The model under review builds one solid part; all positions refer to its coordinate system, in mm. Face numbers are marked on the shaded views. A direction names the side the tool comes from. Round coordinates to 2 decimals unless told otherwise and drop trailing zeros. Order: outer loops, then holes, each group sorted by start corner. A loop starts at its lowest first (then second) coordinate and runs counter-clockwise, first axis right, second up. Notation, with made-up numbers: M 42,29.5 L 57,29.5 A19 cw 57,56.5 Z; hole C -27,43 d8. An arc over 180 degrees is marked long. Answer as a JSON object with one key per item and string values. Group by question number.
1) For the marked faces 1, 2, 3 and 4, list the 3-axis set-ups (+Z, -Z, +X, -X, +Y, -Y) from which the entire face can be reached by the end or side of a thin tool; tool diameter is ignored.
2) The part is to be moulded in two halves that separate along X. For the marked faces 5, 6, 7 and 8, say which applies: +X half, -X half, draft (parallel to the pull), parting line (faces both ways), or undercut.
3) Insertion check: pin 1 Ø10 at (y, z) = (51, 35) entering from +X; pin 2 Ø1.5 at (y, z) = (25.5, 29) entering from +X; pin 3 Ø12 at (x, y) = (45, 34) entering from +Z; pin 4 Ø16 at (y, z) = (40.5, 29.5) entering from -X. Each pin has a flat end and moves straight along its axis. Give the tip position at first contact, or say it passes through.
4) To check wall thickness, follow line 1 (X direction, y = 36.5, z = 26); line 2 (Y direction, x = 50, z = 16.25); line 3 (Z direction, x = 95.5, y = 27). State the ranges of each line that lie inside material, in increasing order.
5) Consider section C-C, the plane z = 32. Write out the cut boundary in (x, y), then the cut area to 3 significant figures.
6) Consider section D-D, the plane y = 45. Write out the cut boundary in (x, z).
7) Consider section B-B, the plane y = 30. Write out the cut boundary in (x, z), then the cut area to 3 significant figures.
8) Consider section A-A, the plane x = 50. Write out the cut boundary in (y, z), then the cut area to 3 significant figures.
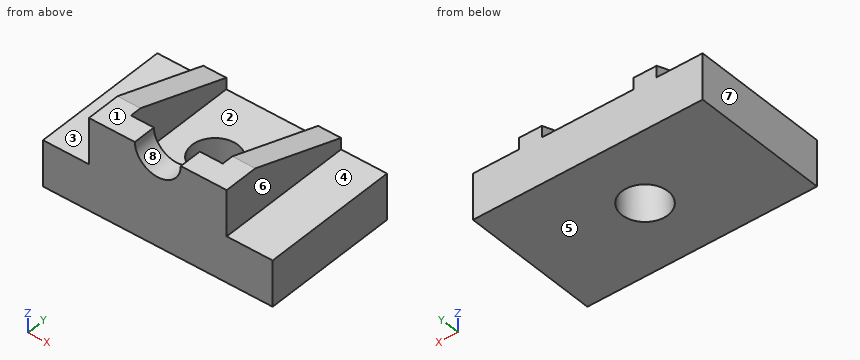
```python
from build123d import *

# Parameters (mm, degrees)
BACK_PLATE_SKETCH_W       = 100
BACK_PLATE_SKETCH_H       = 60
BACK_PLATE_DEPTH          = 20
BORE_20_SKETCH_R          = 10
BORE_20_DEPTH             = 20
NOTCHED_BASE_FLANGE_DEPTH = 10
LEFT_GUSSET_DEPTH         = 10
RIGHT_GUSSET_DEPTH        = 10


with BuildPart() as part:
    # Back Plate Sketch → Back Plate (new body)
    with BuildSketch(Plane.XY):
        with Locations((50, 30)):
            Rectangle(BACK_PLATE_SKETCH_W, BACK_PLATE_SKETCH_H)
    extrude(amount=BACK_PLATE_DEPTH)

    # Bore Ø20 Sketch → Bore Ø20 (cut)
    with BuildSketch(Plane.XY.offset(20)):
        with Locations((50, 30)):
            Circle(BORE_20_SKETCH_R)
    extrude(amount=-BORE_20_DEPTH, mode=Mode.SUBTRACT)

    # Base Flange Sketch → Notched Base Flange (add)
    with BuildSketch(Plane.XZ):
        with BuildLine():
            Line((20, 20), (20, 40))
            Line((20, 40), (40, 40))
            ThreePointArc((40, 40), (50, 30), (60, 40))
            Line((60, 40), (80, 40))
            Line((80, 40), (80, 20))
            Line((80, 20), (20, 20))
        make_face()
    extrude(amount=-NOTCHED_BASE_FLANGE_DEPTH)

    # Left Gusset Sketch → Left Gusset (add)
    with BuildSketch(Plane(origin=(80, 0, 0), x_dir=(0, 0, -1), z_dir=(1, 0, 0))):
        Polygon((-40, 10), (-40, 15), (-25, 60), (-20, 60), (-20, 10), align=None)
    extrude(amount=-LEFT_GUSSET_DEPTH)

    # Right Gusset Sketch → Right Gusset (add)
    with BuildSketch(Plane.ZY.offset(-20)):
        Polygon((40, 10), (40, 15), (25, 60), (20, 60), (20, 10), align=None)
    extrude(amount=-RIGHT_GUSSET_DEPTH)


solid = part.part
```
Results list:
{
 "1": {"face 1": "+Z, +X, -X, +Y, -Y", "face 2": "+Z, +Y", "face 3": "+Z, -X, +Y, -Y", "face 4": "+Z, +X, +Y, -Y"},
 "2": {"face 5": "draft", "face 6": "+X half", "face 7": "-X half", "face 8": "undercut"},
 "3": {"pin 1": "through", "pin 2": "x = 80", "pin 3": "z = 20", "pin 4": "x = 20"},
 "4": {"line 1": "20 to 30, 70 to 80", "line 2": "0 to 20, 40 to 60", "line 3": "0 to 20"},
 "5": {"outline": "M 20,0 L 44,0 L 44,10 L 30,10 L 30,39 L 20,39 Z; M 56,0 L 80,0 L 80,39 L 70,39 L 70,10 L 56,10 Z", "area": "1,060 mm^2"},
 "6": {"outline": "M 0,0 L 100,0 L 100,20 L 80,20 L 80,30 L 70,30 L 70,20 L 30,20 L 30,30 L 20,30 L 20,20 L 0,20 Z"},
 "7": {"outline": "M 0,0 L 40,0 L 40,20 L 30,20 L 30,35 L 20,35 L 20,20 L 0,20 Z; M 60,0 L 100,0 L 100,20 L 80,20 L 80,35 L 70,35 L 70,20 L 60,20 Z", "area": "1,900 mm^2"},
 "8": {"outline": "M 0,0 L 20,0 L 20,20 L 10,20 L 10,30 L 0,30 Z; M 40,0 L 60,0 L 60,20 L 40,20 Z", "area": "900 mm^2"}
}
